```python
from build123d import *

# Parameters (mm, degrees)
SKETCH_1_R      = 1
EXTRUDE_1_DEPTH = 1.2


with BuildPart() as part:
    # 草图1 → 凸台-拉伸1 (new body)
    with BuildSketch(Plane(origin=(0, 0, -1.2), x_dir=(-1, 0, 0), z_dir=(0, 0, -1))):
        with BuildLine():
            Line((-1.25, -16.781097141), (-1.25, -12.362454205))
            ThreePointArc((-1.25, -12.362454205), (0, 10.77), (1.25, -12.362454205))
            Line((1.25, -12.362454205), (1.25, -16.781097141))
            ThreePointArc((1.25, -16.781097141), (4.048302979, -16.309381221), (6.719258119, -15.350728987))
            ThreePointArc((6.719258119, -15.350728987), (6.905510397, -15.201919327), (7.00168518, -14.983780295))
            Line((7.00168518, -14.983780295), (7.468086116, -12.338689143))
            ThreePointArc((7.468086116, -12.338689143), (7.614025765, -11.968002587), (7.893099573, -11.68370571))
            ThreePointArc((7.893099573, -11.68370571), (0, 14.1), (-7.893099573, -11.68370571))
            ThreePointArc((-7.893099573, -11.68370571), (-7.614025765, -11.968002587), (-7.468086116, -12.338689143))
            Line((-7.468086116, -12.338689143), (-7.00168518, -14.983780295))
            ThreePointArc((-7.00168518, -14.983780295), (-6.905510397, -15.201919327), (-6.719258119, -15.350728987))
            ThreePointArc((-6.719258119, -15.350728987), (-4.048302979, -16.309381221), (-1.25, -16.781097141))
        make_face()
        with Locations(Location((-4.25, -13.959261213, 0), (0, 0, 180))):
            Circle(SKETCH_1_R, mode=Mode.SUBTRACT)
        with Locations(Location((4.25, -13.959261213, 0), (0, 0, 180))):
            Circle(SKETCH_1_R, mode=Mode.SUBTRACT)
    extrude(amount=-EXTRUDE_1_DEPTH)


solid = part.part
```
Geometry check sheet. Reference: the model listing, model coordinates, mm. A direction names the side the tool comes from. Give positions to 0.01 mm unless a question says otherwise; leave off trailing zeros. Loops run counter-clockwise (first coordinate to the right, second up) from the corner with the lowest first, then second, coordinate; pieces in that order, holes last. Notation, with made-up numbers: M 42.25,-25.75 L 51.25,-25.75 A34 ccw 51.25,9.25 Z; hole C 18.5,38.5 d2. An arc over 180 degrees is marked long. Write item = value, one per line. Start each with the question number.
1. Section check C-C, the plane z = -0.95. Enter the section's corners in (x, y), plus the area to 3 significant figures.
2. Draft check along Y on faces 1 (the face through (0.49, 10.76, -0.61)), 2 (the face through (-4.01, -16.32, -0.61)), 3 (the face through (1.25, -15, -1)). Enter one of: +Y half, -Y half, draft (parallel to the pull), parting line (faces both ways), or undercut.
3. Section check B-B, the plane x = -5.75. Enter the section's corners in (y, z).
4. Go/stop test with a flat-tipped pin: P1, Ø0.6, axis at y = -15, z = -0.5, coming from the +X side. Record where the tip stops, or that it passes through.
5. Tool access check on faces 4 (the face through (4.033, -12.983, -0.608)), 5 (the face through (-1.25, -15, -1)). Record the directions out of +Z, -Z, +X, -X, +Y, -Y that give a thin tool (end or side, any length) a straight path to the whole face; none if there is none.
6. Section check D-D, the plane x = 0. Enter the section's corners in (y, z), plus the area to 3 significant figures.
7. Section check A-A, the plane y = 2.5. Enter the section's corners in (x, z).
8. Thickness scan on probe 1 along Y at (x, z) = (4.25, -0.25); probe 2 along X at (y, z) = (-0.83, -0.65); probe 3 along Y at (x, z) = (1.5, -0.05). Record the ranges inside material, lowest first.
Values follow:
q1.outline = M -7.89,-11.68 A1 cw -7.47,-12.34 L -7,-14.98 A0.5 ccw -6.72,-15.35 A16 ccw -1.25,-16.78 L -1.25,-12.36 A11.6 cw long 1.25,-12.36 L 1.25,-16.78 A16 ccw 6.72,-15.35 A0.5 ccw 7,-14.98 L 7.47,-12.34 A1 cw 7.89,-11.68 A14.1 ccw long Z; hole C -4.25,-13.96 d2; hole C 4.25,-13.96 d2
q1.area = 225 mm^2
q2.face_1 = undercut
q2.face_2 = -Y half
q2.face_3 = draft
q3.outline = M -15.76,-1.2 L -10.9,-1.2 L -10.9,0 L -15.76,0 Z; M 9.24,-1.2 L 12.87,-1.2 L 12.87,0 L 9.24,0 Z
q4.P1 = 7.05
q5.face_4 = +Z, -Z
q5.face_5 = +Z, -Z, -Y
q6.outline = M 10.77,-1.2 L 14.1,-1.2 L 14.1,0 L 10.77,0 Z
q6.area = 4.00 mm^2
q7.outline = M -13.88,-1.2 L -11.11,-1.2 L -11.11,0 L -13.88,0 Z; M 11.11,-1.2 L 13.88,-1.2 L 13.88,0 L 11.11,0 Z
q8.probe_1 = -16.26 to -14.96, -12.96 to -11.62, 9.96 to 13.44
q8.probe_2 = -14.08 to -11.6, 11.6 to 14.08
q8.probe_3 = -16.76 to -12.33, 10.67 to 14.02
